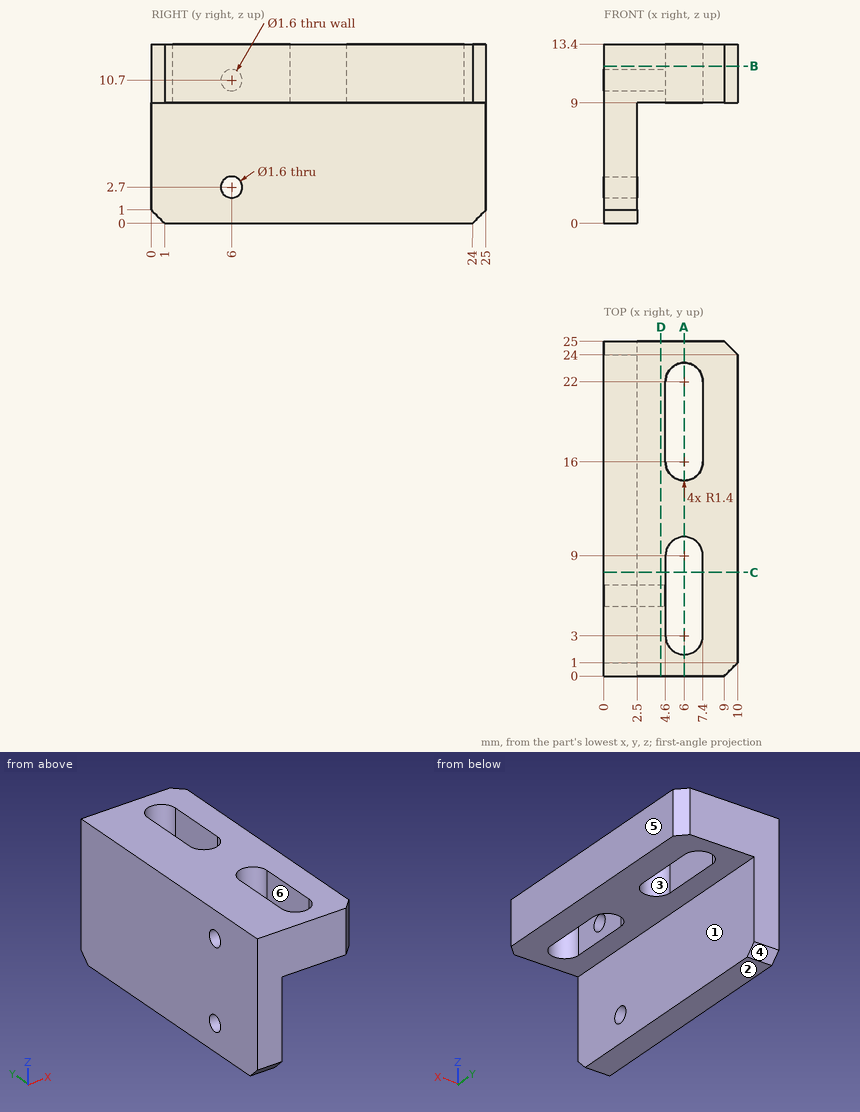
Answer from the drawing. Dimensions are ordinates in mm from the lowest x, y and z of the part. A direction names the side the tool comes from. Give positions to 0.01 mm unless a question says otherwise; leave off trailing zeros. Order: outer loops, then holes, each group sorted by start corner. A loop starts at its lowest first (then second) coordinate and runs counter-clockwise, first axis right, second up. Notation, with made-up numbers: (-16.75, 13.5) - (8.25, 13.5) arc R26 ccw to (8.25, 34.5) - close; hole circle Ø2 at (41, -16). An arc over 180 degrees is marked (long way). One line per item, written item: value. Start each with the question number.
1) A tool of negligible diameter and unlimited length cuts with its end or side. For the marked faces 1, 2 and 3, from which of +Z, -Z, +X, -X, +Y, -Y can it reach the whole face along a straight path? Write none if from no direction.
2) The mould has two halves that part along X. Classify the marked faces 4, 5 and 6: released by +X, released by -X, zero draft, split by the parting line, or undercut.
3) A cutting plane is placed at A-A on x = 6. Give the vertices of the cut face in (y, z).
4) A cutting plane is placed at C-C on y = 7.75. Give the vertices of the cut face in (x, z).
5) A cutting plane is placed at D-D on x = 4.25. Give the vertices of the cut face in (y, z).
6) Given pin 1 Ø1.5 at (y, z) = (21, 11) entering from -X; pin 2 Ø4.5 at (y, z) = (18.5, 5.5) entering from +X, each flat-ended and moving along its own axis, determine where each tip first touches the part or whether it passes through.
7) Find the intervals of material crossed by L1, parallel to Y at x = 2, z = 10.7; L2, parallel to Y at x = 5.25, z = 12; L3, parallel to Y at x = 7, z = 11, in increasing order.
8) A cutting plane is placed at B-B on z = 11.75. Give the vertices of the cut face in (x, y).
Answer sheet:
1. face 1: -Z, +X, +Y, -Y
1. face 2: -Z, +X, -X, +Y, -Y
1. face 3: +Z, -Z
2. face 4: zero draft
2. face 5: released by +X
2. face 6: undercut
3. outline: (0, 9) - (1.6, 9) - (1.6, 13.4) - (0, 13.4) - close; (10.4, 9) - (14.6, 9) - (14.6, 13.4) - (10.4, 13.4) - close; (23.4, 9) - (25, 9) - (25, 13.4) - (23.4, 13.4) - close
4. outline: (0, 0) - (2.5, 0) - (2.5, 9) - (4.6, 9) - (4.6, 13.4) - (0, 13.4) - close; (7.4, 9) - (10, 9) - (10, 13.4) - (7.4, 13.4) - close
5. outline: (0, 9) - (25, 9) - (25, 13.4) - (0, 13.4) - close; hole circle Ø1.6 at (6, 10.7)
6. pin 1: stops at x = 0
6. pin 2: stops at x = 2.5
7. L1: y = 0 to 5.2, 6.8 to 25
7. L2: y = 0 to 1.82, 10.18 to 14.82, 23.18 to 25
7. L3: y = 0 to 2.02, 9.98 to 15.02, 22.98 to 25
8. outline: (0, 0) - (9, 0) - (10, 1) - (10, 24) - (9, 25) - (0, 25) - close; hole (4.6, 3) arc R1.4 ccw to (7.4, 3) - (7.4, 9) arc R1.4 ccw to (4.6, 9) - close; hole (4.6, 16) arc R1.4 ccw to (7.4, 16) - (7.4, 22) arc R1.4 ccw to (4.6, 22) - close
